Part model, mm, in its own coordinate system. Face numbers are marked on the shaded views. A direction names the side the tool comes from. Round coordinates to 2 decimals unless told otherwise and drop trailing zeros. Loops run counter-clockwise (first coordinate to the right, second up) from the corner with the lowest first, then second, coordinate; pieces in that order, holes last. Notation, with made-up numbers: (46, 46.25) - (78, 46.25) arc R21 cw to (78, 76.25) - close; hole circle Ø1 at (88.25, 64.5). An arc over 180 degrees is marked (long way). Put each result on its own line as item: value.
from build123d import *

# Parameters (mm, degrees)
BOSS_EXTRUDE1_DEPTH   = 25
BOSS_EXTRUDE2_DEPTH   = 27.5
CUT_EXTRUDE1_DEPTH    = 82.952730278
SKETCH4_R             = 6.5
SKETCH4_R_2           = 3
CUT_EXTRUDE2_DEPTH    = 82.95273041
M6_TAPPED_HOLE1_D     = 5
M6_TAPPED_HOLE1_DEPTH = 17
M6_TAPPED_HOLE1_TIP   = 1.502151548


with BuildPart() as part:
    # Sketch1 → Boss-Extrude1 (new, symmetric)
    with BuildSketch(Plane.XY):
        with BuildLine():
            Line((-62, 0), (-30, 0))
            ThreePointArc((-30, 0), (0, 30), (30, 0))
            Line((30, 0), (62, 0))
            ThreePointArc((62, 0), (0, 62), (-62, 0))
        make_face()
    extrude(amount=BOSS_EXTRUDE1_DEPTH, both=True)

    # Sketch2 → Boss-Extrude2 (add, symmetric)
    with BuildSketch(Plane.XY):
        with BuildLine():
            Line((-50, 0), (-30, 0))
            ThreePointArc((-30, 0), (0, 30), (30, 0))
            Line((30, 0), (50, 0))
            ThreePointArc((50, 0), (0, 50), (-50, 0))
        make_face()
    extrude(amount=BOSS_EXTRUDE2_DEPTH, both=True)

    # Sketch3 → Cut-Extrude1 (cut, through all)
    with BuildSketch(Plane(origin=(0, 16, 0), x_dir=(1, 0, 0), z_dir=(0, 1, 0))):
        with BuildLine():
            Line((-75, 17), (-50, 17))
            ThreePointArc((-50, 17), (-33, 0), (-50, -17))
            Line((-50, -17), (-75, -17))
            Line((-75, -17), (-75, 17))
        make_face()
        with BuildLine():
            Line((75, -17), (50, -17))
            ThreePointArc((50, -17), (33, 0), (50, 17))
            Line((50, 17), (75, 17))
            Line((75, 17), (75, -17))
        make_face()
    extrude(amount=CUT_EXTRUDE1_DEPTH, mode=Mode.SUBTRACT)

    # Sketch4 → Cut-Extrude2 (cut, through all)
    with BuildSketch(Plane(origin=(0, 16, 0), x_dir=(1, 0, 0), z_dir=(0, 1, 0))):
        with Locations(Location((-50, 0, 0), (0, 0, 270))):
            Circle(SKETCH4_R)
        with Locations(Location((-50, 12, 0), (0, 0, 270))):
            Circle(SKETCH4_R_2)
        with Locations(Location((50, 0, 0), (0, 0, 90))):
            Circle(SKETCH4_R)
        with Locations(Location((50, -12, 0), (0, 0, 270))):
            Circle(SKETCH4_R_2)
    extrude(amount=-CUT_EXTRUDE2_DEPTH, mode=Mode.SUBTRACT)

    # M6 Tapped Hole1
    with Locations(Plane.XY.offset(27.5)):
        with Locations((0, 40)):
            Hole(M6_TAPPED_HOLE1_D / 2, depth=M6_TAPPED_HOLE1_DEPTH)
            with Locations((0, 0, -(M6_TAPPED_HOLE1_DEPTH + M6_TAPPED_HOLE1_TIP / 2))):  # 118° drill point
                Cone(0, M6_TAPPED_HOLE1_D / 2, M6_TAPPED_HOLE1_TIP, mode=Mode.SUBTRACT)


solid = part.part
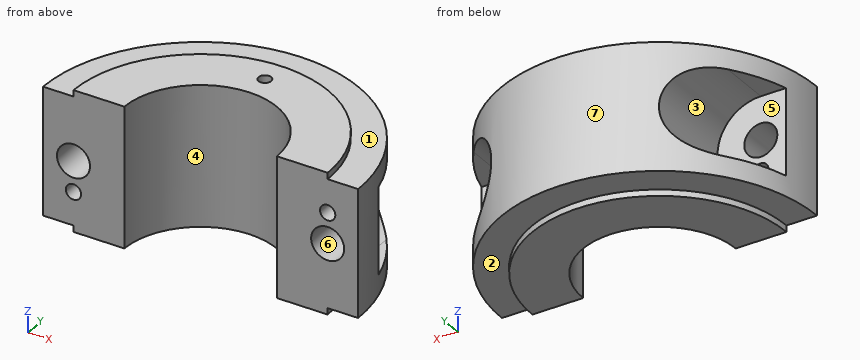
1. Band-saw the part on D-D (z = -12). List the corners of the cut face in (x, y).
A:
outline: (-62, 0) - (-53, 0) - (-53, 16) - (-59.9, 16) arc R62 ccw to start; (-47, 0) - (-30, 0) arc R30 cw to (30, 0) - (62, 0) arc R62 ccw to (59.9, 16) - (37.96, 16) - (37.96, 49.02) arc R62 ccw to (-37.96, 49.02) - (-37.96, 16) - (-47, 16) - close
2. Pin check, flat tips, straight feed: P1, Ø11.5, axis at x = -50, z = 0, coming from the +Y side; P2, Ø1, axis at y = 17.5, z = 1, coming from the +X side; P3, Ø3, axis at y = 9.5, z = 15.5, coming from the -X side; P4, Ø5, axis at x = 53, y = 21.5, coming from the +Z side. Stop position of each tip, or through.
A:
P1: passes through
P2: stops at x = 33.07
P3: stops at x = -61.48
P4: stops at z = 25
3. Band-saw the part on C-C (z = 20.5). List the corners of the cut face in (x, y), plus the area to 3 significant figures.
A:
outline: (-62, 0) - (-30, 0) arc R30 cw to (30, 0) - (62, 0) arc R62 ccw to start; hole circle Ø5 at (0, 40)
area: 4,600 mm²
4. Tool access for the marked faces 1, 2 and 3: list every direction of +Z, -Z, +X, -X, +Y, -Y with a clear straight run to the whole face (end or side of a thin tool).
A:
face 1: +Z, +Y
face 2: -Z, +Y
face 3: -X, +Y
5. Two-plate mould, pull along X, no slides. Class the marked faces 4, 5, 6 and 7: pulls with the +X half, pulls with the -X half, needs draft (parallel to the pull), parting line crosses it, or undercut.
A:
face 4: undercut
face 5: needs draft
face 6: undercut
face 7: parting line crosses it
6. Probe line 1 along X through (y, z) = (11, 0); line 2 along X through (y, z) = (8, 12); line 3 along X through (y, z) = (4, 12). List the from-to ranges inside material, lowest first. Write a range as [from, to].
A:
line 1: x = [-61.02, -56.5], [-43.5, -27.91], [27.91, 43.5], [56.5, 61.02]
line 2: x = [-61.48, -28.91], [28.91, 47], [53, 61.48]
line 3: x = [-61.87, -29.73], [29.73, 47], [53, 61.87]
7. Band-saw the part on A-A (z = 0). List the corners of the cut face in (x, y), plus the area to 3 significant figures.
A:
outline: (-62, 0) - (-56.5, 0) - (-56.5, 16) - (-59.9, 16) arc R62 ccw to start; (-43.5, 0) - (-30, 0) arc R30 cw to (30, 0) - (43.5, 0) - (43.5, 16) - (33, 16) - (33, 52.49) arc R62 ccw to (-33, 52.49) - (-33, 16) - (-43.5, 16) - close; (56.5, 0) - (62, 0) arc R62 ccw to (59.9, 16) - (56.5, 16) - close
area: 2,970 mm²
8. Band-saw the part on B-B (y = 12). List the corners of the cut face in (x, z).
A:
outline: (-60.83, -25) - (-48.54, -25) - (-48.54, -27.5) - (-27.5, -27.5) - (-27.5, 27.5) - (-48.54, 27.5) - (-48.54, 25) - (-60.83, 25) - close; (27.5, -27.5) - (48.54, -27.5) - (48.54, -25) - (60.83, -25) - (60.83, 25) - (48.54, 25) - (48.54, 27.5) - (27.5, 27.5) - close; hole circle Ø13 at (-50, 0); hole circle Ø6 at (-50, -12); hole circle Ø13 at (50, 0); hole circle Ø6 at (50, 12)
